Work out the finished part from the listing and answer in its coordinate system (mm). Give positions to 0.01 mm unless a question says otherwise; leave off trailing zeros. Loops run counter-clockwise (first coordinate to the right, second up) from the corner with the lowest first, then second, coordinate; pieces in that order, holes last. Notation, with made-up numbers: M 29.25,55 L 50.25,55 A22 ccw 50.25,80 Z; hole C -37.75,55.5 d10. An arc over 180 degrees is marked long. Write item = value, one per line. Start each with the question number.
1. Section B-B on x = -7 is taken. Determine the outline of the cut face in (y, z), plus the area to 3 significant figures.
2. Consider L1, parallel to Y at x = 0, z = 50; L2, parallel to X at y = -2, z = 54.5; L3, parallel to X at y = -0.5, z = 17. Determine where each line is inside the solid, lowest interval first. Write a range as [from, to].
3. Section A-A on z = 20.5 is taken. Determine the outline of the cut face in (x, y), plus the area to 3 significant figures.
4. Flat-ended cylindrical pins translate along their axes: pin 1 Ø4 at (x, z) = (-9.5, 36) entering from -Y; pin 2 Ø5 at (x, z) = (-9.5, 15) entering from -Y; pin 3 Ø5 at (x, z) = (9.5, 52.5) entering from +Y. Find the tip coordinate at first contact, or state that the pin passes through.
5. Section C-C on y = -5.5 is taken. Determine the outline of the cut face in (x, z), plus the area to 3 significant figures.
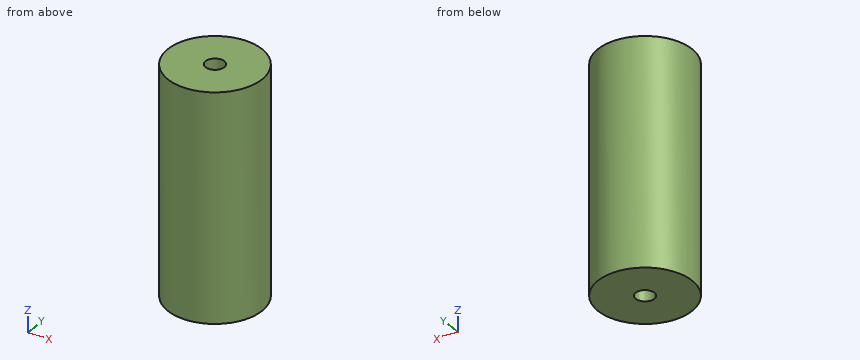
```python
from build123d import *

# Parameters (mm, degrees)
SKETCH_1_R             = 12.5
BOSS_EXTRUDE_1_DEPTH   = 60
M6_TAPPED_HOLE_1_D     = 5
M6_TAPPED_HOLE_1_DEPTH = 15
M6_TAPPED_HOLE_1_TIP   = 1.502151548
M6_TAPPED_HOLE_2_D     = 5
M6_TAPPED_HOLE_2_DEPTH = 15
M6_TAPPED_HOLE_2_TIP   = 1.502151548


with BuildPart() as part:
    # Sketch 1 → Boss-Extrude 1 (new body)
    with BuildSketch(Plane.XY):
        Circle(SKETCH_1_R)
    extrude(amount=BOSS_EXTRUDE_1_DEPTH)

    # M6 Tapped Hole 1
    with Locations(Plane.XY.offset(60)):
        with Locations((0, 0)):
            Hole(M6_TAPPED_HOLE_1_D / 2, depth=M6_TAPPED_HOLE_1_DEPTH)
            with Locations((0, 0, -(M6_TAPPED_HOLE_1_DEPTH + M6_TAPPED_HOLE_1_TIP / 2))):  # 118° drill point
                Cone(0, M6_TAPPED_HOLE_1_D / 2, M6_TAPPED_HOLE_1_TIP, mode=Mode.SUBTRACT)

    # M6 Tapped Hole 2
    with Locations(Plane(origin=(0, 0, 0), x_dir=(-1, 0, 0), z_dir=(0, 0, -1))):
        with Locations((0, 0)):
            Hole(M6_TAPPED_HOLE_2_D / 2, depth=M6_TAPPED_HOLE_2_DEPTH)
            with Locations((0, 0, -(M6_TAPPED_HOLE_2_DEPTH + M6_TAPPED_HOLE_2_TIP / 2))):  # 118° drill point
                Cone(0, M6_TAPPED_HOLE_2_D / 2, M6_TAPPED_HOLE_2_TIP, mode=Mode.SUBTRACT)


solid = part.part
```
Verdict:
q1.outline = M -10.36,0 L 10.36,0 L 10.36,60 L -10.36,60 Z
q1.area = 1,240 mm2
q2.L1 = [-12.5, -2.5], [2.5, 12.5]
q2.L2 = [-12.34, -1.5], [1.5, 12.34]
q2.L3 = [-12.49, 12.49]
q3.outline = C 0,0 d25
q3.area = 491 mm2
q4.pin_1 = -10
q4.pin_2 = -10.36
q4.pin_3 = 10.36
q5.outline = M -11.22,0 L 11.22,0 L 11.22,60 L -11.22,60 Z
q5.area = 1,350 mm2
